```python
from build123d import *

# Parameters (mm, degrees)
FRONT_EAR_PROFILE_SKETCH_R = 5
FRONT_EAR_PLATE_DEPTH      = 10
BRIDGE_WALL_SKETCH_W       = 10
BRIDGE_WALL_SKETCH_H       = 42
BRIDGE_WALL_DEPTH          = 60
REAR_EAR_PROFILE_SKETCH_R  = 5
REAR_EAR_PLATE_DEPTH       = 10
COLLAR_SKETCH_26_R         = 20
SHANK_COLLAR_26_DEPTH      = 25
COLLAR_FILLET_R3_R         = 3
PIN_SHANK_SKETCH_R         = 12.5
PIN_SHANK_DEPTH            = 33
SHANK_END_FILLET_R3_R      = 3


with BuildPart() as part:
    # Front Ear Profile Sketch → Front Ear Plate (new body)
    with BuildSketch(Plane.XY):
        with BuildLine():
            Line((0, 0), (68, 0))
            ThreePointArc((68, 0), (98, 30), (68, 60))
            Line((68, 60), (0, 60))
            Line((0, 60), (0, 0))
        make_face()
        with Locations((68, 30)):
            Circle(FRONT_EAR_PROFILE_SKETCH_R, mode=Mode.SUBTRACT)
        with Locations((48, 30)):
            Circle(FRONT_EAR_PROFILE_SKETCH_R, mode=Mode.SUBTRACT)
    extrude(amount=FRONT_EAR_PLATE_DEPTH)

    # Bridge Wall Sketch → Bridge Wall (add)
    with BuildSketch(Plane(origin=(0, 60, 0), x_dir=(1, 0, 0), z_dir=(0, 1, 0))):
        with Locations((5, 21)):
            Rectangle(BRIDGE_WALL_SKETCH_W, BRIDGE_WALL_SKETCH_H)
    extrude(amount=-BRIDGE_WALL_DEPTH)

    # Rear Ear Profile Sketch → Rear Ear Plate (add)
    with BuildSketch(Plane(origin=(0, 0, -42), x_dir=(-1, 0, 0), z_dir=(0, 0, -1))):
        with BuildLine():
            Line((-10, 60), (-68, 60))
            ThreePointArc((-68, 60), (-98, 30), (-68, 0))
            Line((-68, 0), (-10, 0))
            Line((-10, 0), (-10, 60))
        make_face()
        with Locations(Location((-68, 30, 0), (0, 0, 180))):
            Circle(REAR_EAR_PROFILE_SKETCH_R, mode=Mode.SUBTRACT)
        with Locations(Location((-48, 30, 0), (0, 0, 180))):
            Circle(REAR_EAR_PROFILE_SKETCH_R, mode=Mode.SUBTRACT)
    extrude(amount=-REAR_EAR_PLATE_DEPTH)

    # Collar Sketch Ø26 → Shank Collar Ø26 (add)
    with BuildSketch(Plane.ZY):
        with Locations((-16, 30)):
            Circle(COLLAR_SKETCH_26_R)
    extrude(amount=SHANK_COLLAR_26_DEPTH)

    # Collar Fillet R3
    collar_fillet_r3_edges = [part.edges().sort_by_distance(p)[0] for p in [
        (0, 30, -36),
    ]]
    fillet(collar_fillet_r3_edges, radius=COLLAR_FILLET_R3_R)

    # Pin Shank Sketch → Pin Shank (add)
    with BuildSketch(Plane.ZY.offset(25)):
        with Locations((-16, 30)):
            Circle(PIN_SHANK_SKETCH_R)
    extrude(amount=PIN_SHANK_DEPTH)

    # Shank End Fillet R3
    shank_end_fillet_r3_edges = [part.edges().sort_by_distance(p)[0] for p in [
        (-58, 30, -28.5),
    ]]
    fillet(shank_end_fillet_r3_edges, radius=SHANK_END_FILLET_R3_R)


solid = part.part
```
The listing builds one solid part. Answer for the finished solid, in the listing's coordinates (mm). A direction names the side the tool comes from. Coordinates: 2 decimals unless noted, no trailing zeros. Loops run counter-clockwise (first coordinate to the right, second up) from the corner with the lowest first, then second, coordinate; pieces in that order, holes last. Notation, with made-up numbers: M 18,27 L 77,27 A19 ccw 77,55 Z; hole C -5,-17 d8. An arc over 180 degrees is marked long. Answer as a JSON object with one key per item and string values. Group by question number.
Item 1: Each of these flat-tipped pins is pushed along its axis until it touches: P1, Ø3, axis at x = -18.5, z = -16, coming from the -Y side; P2, Ø1, axis at x = -34, z = -18.5, coming from the +Y side; P3, Ø10, axis at y = 33, z = -12, coming from the +X side. Where does it stop, or does it pass through?
Item 2: Section A-A (x = 48) is taken. Write down the section's boundary in (y, z).
Item 3: Determine the mould class of faces 4 (the face through (97.993, 29.34, 4.93)), 5 (the face through (-58, 30, -16)), 6 (the face through (48, 24, 10)), 7 (the face through (44, 27, 5)) for opening direction X: +X half, -X half, draft (parallel to the pull), parting line (faces both ways), or undercut.
Item 4: Section D-D (y = 4) is taken. Write down the section's boundary in (x, z).
Item 5: Section B-B (z = -16) is taken. Write down the section's boundary in (x, y), and give its area (4 significant figures).
Item 6: Section C-C (y = 30) is taken. Give the number of separate pieces and of enclosed holes in the cut face, and give its area (4 significant figures).
Item 7: Consider L1, parallel to Y at x = 68, z = -35.75; L2, parallel to Z at x = 17, y = 14.5; L3, parallel to X at y = 27, z = -16. Determine where each line is inside the solid, lowest interval first.
Item 8: Which of the six approach directions +Z, -Z, +X, -X, +Y, -Y give full straight-line access (tool end or side, diameter ignored) to faces 1 (the face through (97.993, 30.66, -37.07)), 2 (the face through (-13.85, 49.83, -18.6)), 3 (the face through (10, 30, -16))?
Solved:
{
 "1": {"P1": "stops at y = 10", "P2": "stops at y = 42.34", "P3": "stops at x = 10"},
 "2": {"outline": "M 0,-42 L 25,-42 L 25,-32 L 0,-32 Z; M 0,0 L 25,0 L 25,10 L 0,10 Z; M 35,-42 L 60,-42 L 60,-32 L 35,-32 Z; M 35,0 L 60,0 L 60,10 L 35,10 Z"},
 "3": {"face 4": "+X half", "face 5": "-X half", "face 6": "draft", "face 7": "undercut"},
 "4": {"outline": "M 0,-42 L 82.97,-42 L 82.97,-32 L 10,-32 L 10,0 L 82.97,0 L 82.97,10 L 0,10 Z"},
 "5": {"outline": "M -58,20.5 A3 ccw -55,17.5 L -25,17.5 L -25,10 L -3,10 A3 cw 0,7 L 0,0 L 10,0 L 10,60 L 0,60 L 0,53 A3 cw -3,50 L -25,50 L -25,42.5 L -55,42.5 A3 ccw -58,39.5 Z", "area": "2,425 mm2"},
 "6": {"separate pieces": "5", "enclosed holes": "0", "area": "3,705 mm2"},
 "7": {"L1": "y = 0 to 25, 35 to 60", "L2": "z = -42 to -32, 0 to 10", "L3": "x = -58 to 10"},
 "8": {"face 1": "+Z, -Z, +X", "face 2": "-X", "face 3": "+X, +Y, -Y"}
}
